Part model, mm, in its own coordinate system. Face numbers are marked on the shaded views. A direction names the side the tool comes from. Give positions to 0.01 mm unless a question says otherwise; leave off trailing zeros. Write each loop counter-clockwise with the first axis right and the second up, starting at its lowest first coordinate (ties: lowest second). Pieces come first, ordered by that corner, then holes. Notation, with made-up numbers: M 75,28 L 104,28 A14 cw 104,44 Z; hole C 3.25,75.25 d10. An arc over 180 degrees is marked long. Answer as CSV lines item,"result". Start each with the question number.
Item 1: Band-saw the part on D-D, the plane y = 42.5. List the corners of the cut face in (x, z).
Item 2: 3-axis set-ups, long thin cutter, end or side, ignore diameter. For the marked faces 1, 2 and 3: which of +Z, -Z, +X, -X, +Y, -Y reach the whole face in a straight line?
Item 3: Band-saw the part on B-B, the plane z = 75. List the corners of the cut face in (x, y), then the cut area to 3 significant figures.
Item 4: Two-plate mould, pull along Y, no slides. Class the marked faces 4, 5, 6 and 7: +Y half, -Y half, draft (parallel to the pull), parting line (faces both ways), or undercut.
Item 5: Band-saw the part on C-C, the plane x = 57.5. List the corners of the cut face in (y, z), then the cut area to 3 significant figures.
Item 6: Pin check, flat tips, straight feed: pin 1 (24 mm diameter, centred on y = 33, z = 46.5, fed in from +X); pin 2 (12 mm diameter, centred on x = 70, z = 75, fed in from -Y); pin 3 (23 mm diameter, centred on x = 70, z = 25, fed in from +Y). Stop position of each tip, or through.
Item 7: Wall check: L1, parallel to X at y = -6, z = 75; L2, parallel to Y at x = 57, z = 11.5; L3, parallel to Z at x = 14, y = 84. Give the ranges that are in metal, low to high. Write a range as from..to.
Item 8: Band-saw the part on A-A, the plane x = 76. List the corners of the cut face in (y, z).
from build123d import *

# Parameters (mm, degrees)
BOSS_EXTRUDE1_DEPTH = 100
SKETCH2_R           = 10
CUT_EXTRUDE1_DEPTH  = 500
CUT_EXTRUDE2_DEPTH  = 500


with BuildPart() as part:
    # Sketch1 → Boss-Extrude1 (new body)
    with BuildSketch(Plane.XY):
        Polygon((0, 0), (100, 0), (100, -15), (-15, -15), (-15, 95), (100, 95), (100, 80), (0, 80), align=None)
    extrude(amount=BOSS_EXTRUDE1_DEPTH)

    # Sketch2 → Cut-Extrude1 (cut)
    with BuildSketch(Plane(origin=(0, 95, 0), x_dir=(1, 0, 0), z_dir=(0, 1, 0))):
        with Locations(Location((20, -25, 0), (0, 0, 270))):
            Circle(SKETCH2_R)
        with Locations(Location((70, -25, 0), (0, 0, 270))):
            Circle(SKETCH2_R)
        with Locations(Location((20, -75, 0), (0, 0, 270))):
            Circle(SKETCH2_R)
        with Locations(Location((70, -75, 0), (0, 0, 270))):
            Circle(SKETCH2_R)
    extrude(amount=-CUT_EXTRUDE1_DEPTH, mode=Mode.SUBTRACT)

    # Sketch3 → Cut-Extrude2 (cut)
    with BuildSketch(Plane(origin=(0, 0, 0), x_dir=(0, 0, -1), z_dir=(1, 0, 0))):
        with BuildLine():
            Line((-69.989356501, 46.65904216), (-50.973619408, 62.245711909))
            ThreePointArc((-50.973619408, 62.245711909), (-39.615619928, 61.120144392), (-40.741187444, 49.762144912))
            Line((-40.741187444, 49.762144912), (-59.756924537, 34.175475163))
            ThreePointArc((-59.756924537, 34.175475163), (-71.114924017, 35.30104268), (-69.989356501, 46.65904216))
        make_face()
        with BuildLine():
            Line((-47.157034179, 25.869701183), (-29.932799149, 44.934026231))
            ThreePointArc((-29.932799149, 44.934026231), (-18.599572272, 45.508702041), (-18.024896462, 34.175475163))
            Line((-18.024896462, 34.175475163), (-35.249131491, 15.111150116))
            ThreePointArc((-35.249131491, 15.111150116), (-46.582358369, 14.536474306), (-47.157034179, 25.869701183))
        make_face()
    extrude(amount=-CUT_EXTRUDE2_DEPTH, mode=Mode.SUBTRACT)


solid = part.part
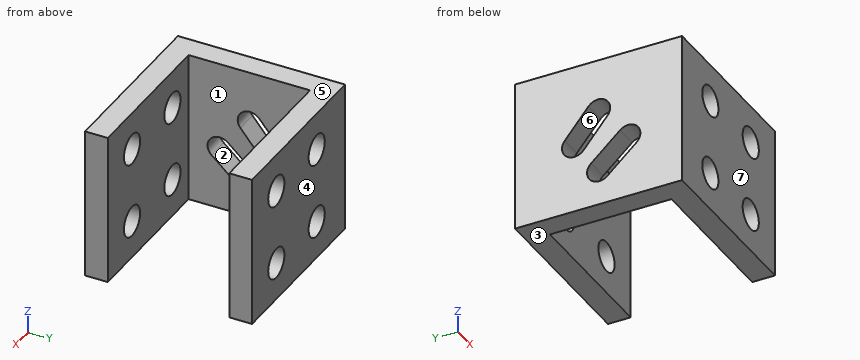
Output:
1,outline,"M -15,0 L 0,0 L 0,16.51 L -15,16.51 Z; M -15,32.13 L 0,32.13 L 0,49.6 L -15,49.6 Z; M -15,72.67 L 0,72.67 L 0,100 L -15,100 Z"
2,face 1,"+Z, -Z, +X"
2,face 2,"+X, -X"
2,face 3,"-Z, +X, -X, +Y, -Y"
3,outline,"M -15,-15 L 10,-15 L 10,0 L 0,0 L 0,80 L 10,80 L 10,95 L -15,95 Z; M 30,-15 L 60,-15 L 60,0 L 30,0 Z; M 30,80 L 60,80 L 60,95 L 30,95 Z; M 80,-15 L 100,-15 L 100,0 L 80,0 Z; M 80,80 L 100,80 L 100,95 L 80,95 Z"
3,area,"3,450 mm²"
4,face 4,"+Y half"
4,face 5,"draft"
4,face 6,"undercut"
4,face 7,"-Y half"
5,outline,"M -15,0 L 0,0 L 0,100 L -15,100 Z; M 80,0 L 95,0 L 95,100 L 80,100 Z"
5,area,"3,000 mm²"
6,pin 1,"x = 0"
6,pin 2,"through"
6,pin 3,"y = 95"
7,L1,"-15..10, 30..60, 80..100"
7,L2,"-15..0, 80..95"
7,L3,"0..17, 33..67, 83..100"
8,outline,"M -15,0 L 0,0 L 0,17 L -15,17 Z; M -15,33 L 0,33 L 0,67 L -15,67 Z; M -15,83 L 0,83 L 0,100 L -15,100 Z; M 80,0 L 95,0 L 95,17 L 80,17 Z; M 80,33 L 95,33 L 95,67 L 80,67 Z; M 80,83 L 95,83 L 95,100 L 80,100 Z"
